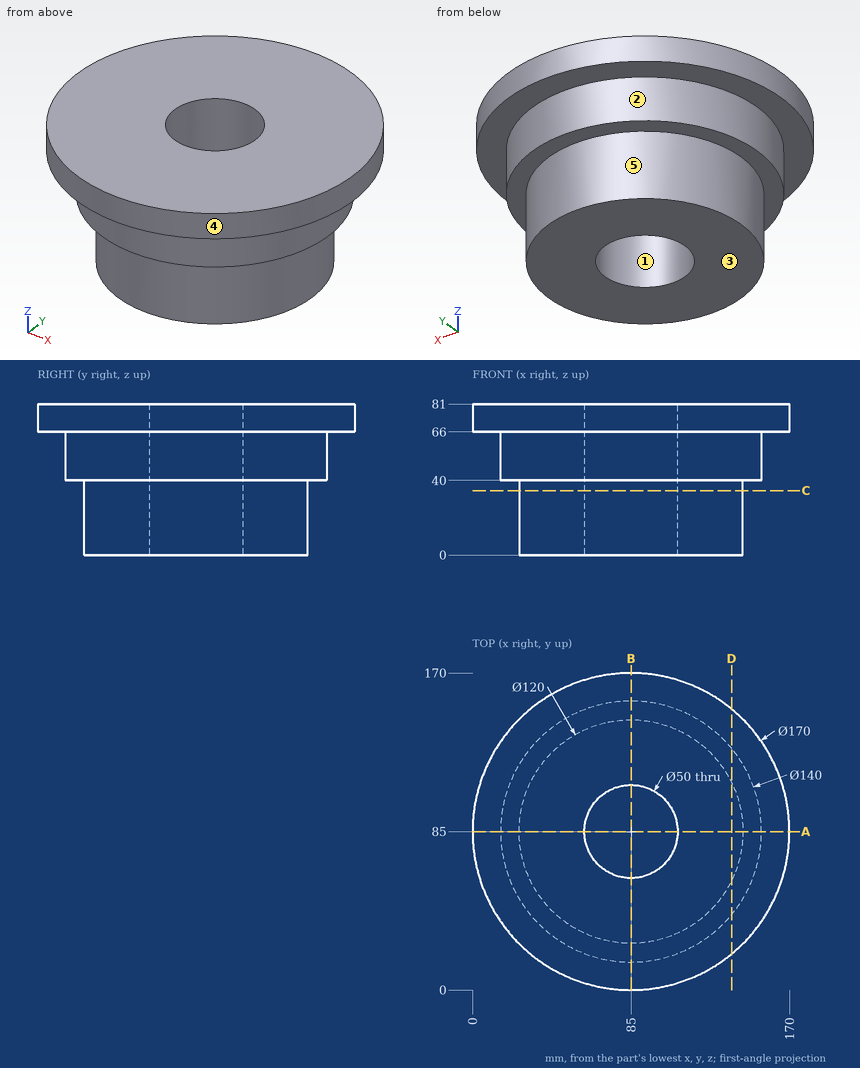
Study the drawing (mm; zero at the part's minimum x, y, z) and answer. A direction names the side the tool comes from. Give positions to 0.01 mm unless a question says otherwise; leave off trailing zeros. Write each loop counter-clockwise with the first axis right and the second up, starting at its lowest first coordinate (ties: lowest second). Pieces come first, ordered by that corner, then holes. Notation, with made-up numbers: (13.5, 56) -> (34.5, 56) arc R15 ccw to (34.5, 77) -> close; hole circle Ø10 at (86, 18). An arc over 180 degrees is marked (long way). Answer in a Markdown table with one row per item.
1) A tool of negligible diameter and unlimited length cuts with its end or side. For the marked faces 4 and 5, from which of +Z, -Z, +X, -X, +Y, -Y can it reach the whole face along a straight path? Write none if from no direction.
Results list:
| item | result |
|---|---|
| face 4 | +Z, -Z |
| face 5 | -Z |
2) Section D-D on x = 139 is taken. Give the vertices of the cut face in (y, z).
Results list:
| item | result |
|---|---|
| outline | (19.36, 66) -> (40.46, 66) -> (40.46, 40) -> (58.85, 40) -> (58.85, 0) -> (111.15, 0) -> (111.15, 40) -> (129.54, 40) -> (129.54, 66) -> (150.64, 66) -> (150.64, 81) -> (19.36, 81) -> close |
3) Each of these flat-tipped pins is pushed along its axis until it touches: pin 1 Ø12 at (y, z) = (38, 57) entering from +X; pin 2 Ø2 at (x, y) = (108.5, 86.5) entering from -Z; pin 3 Ø12 at (x, z) = (35, 55) entering from +Y; pin 4 Ø8 at (x, z) = (46, 10) entering from +Y. Where does it stop, or does it pass through?
Results list:
| item | result |
|---|---|
| pin 1 | x = 141.74 |
| pin 2 | through |
| pin 3 | y = 139.44 |
| pin 4 | y = 133.73 |
4) Straight lines are drawn through the part: line 1 (Y direction, x = 85, z = 28); line 2 (Z direction, x = 120.5, y = 26); line 3 (X direction, y = 105.5, z = 55.5). For each, find the intervals that lie inside material, in ascending order. Write a range as [from, to].
Results list:
| item | result |
|---|---|
| line 1 | [25, 60], [110, 145] |
| line 2 | [40, 81] |
| line 3 | [18.07, 70.69], [99.31, 151.93] |
5) Section A-A on y = 85 is taken. Give the vertices of the cut face in (x, z), plus the area to 3 significant figures.
Results list:
| item | result |
|---|---|
| outline | (0, 66) -> (15, 66) -> (15, 40) -> (25, 40) -> (25, 0) -> (60, 0) -> (60, 81) -> (0, 81) -> close; (110, 0) -> (145, 0) -> (145, 40) -> (155, 40) -> (155, 66) -> (170, 66) -> (170, 81) -> (110, 81) -> close |
| area | 6,940 mm^2 |
6) Determine the mould class of the marked faces 1, 2 and 3 for opening direction X: released by +X, released by -X, zero draft, split by the parting line, or undercut.
Results list:
| item | result |
|---|---|
| face 1 | undercut |
| face 2 | split by the parting line |
| face 3 | zero draft |
7) Section C-C on z = 34.5 is taken. Give the vertices of the cut face in (x, y), plus the area to 3 significant figures.
Results list:
| item | result |
|---|---|
| outline | circle Ø120 at (85, 85); hole circle Ø50 at (85, 85) |
| area | 9,350 mm^2 |
